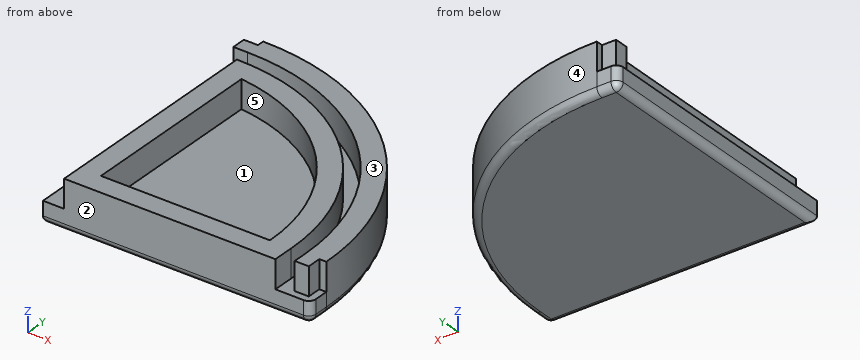
from build123d import *

# Parameters (mm, degrees)
BOSS_EXTRUDE1_DEPTH = 1.5
BOSS_EXTRUDE2_DEPTH = 2
FILETE1_R           = 0.5


with BuildPart() as part:
    # Sketch1 → Boss-Extrude1 (new body)
    with BuildSketch(Plane.XY):
        with BuildLine():
            Line((0, 0), (0, 19))
            Line((0, 19), (1.5, 19))
            ThreePointArc((1.5, 19), (13.874368671, 13.874368671), (19, 1.5))
            Line((19, 1.5), (19, 0))
            Line((19, 0), (0, 0))
        make_face()
    extrude(amount=BOSS_EXTRUDE1_DEPTH)

    # Sketch2 → Boss-Extrude2 (add)
    # profile 1 of 2: a face of its own
    with BuildSketch(Plane.XY.offset(1.5)):
        with BuildLine():
            Line((1.5, 19), (1.5, 18.5))
            Line((1.5, 18.5), (0.5, 18.5))
            Line((0.5, 18.5), (0.5, 17.5))
            Line((0.5, 17.5), (1.5, 17.5))
            ThreePointArc((1.5, 17.5), (12.813708499, 12.813708499), (17.5, 1.5))
            Line((17.5, 1.5), (17.5, 0.5))
            Line((17.5, 0.5), (18.5, 0.5))
            Line((18.5, 0.5), (18.5, 1.5))
            Line((18.5, 1.5), (19, 1.5))
            ThreePointArc((19, 1.5), (13.874368671, 13.874368671), (1.5, 19))
        make_face()
    # profile 2 of 2: a face of its own
    with BuildSketch(Plane.XY.offset(1.5)):
        with BuildLine():
            Line((1.5, 16.5), (1.5, 0))
            Line((1.5, 0), (16.5, 0))
            Line((16.5, 0), (16.5, 1.5))
            ThreePointArc((16.5, 1.5), (12.106601718, 12.106601718), (1.5, 16.5))
        make_face()
        with BuildLine():
            Line((3, 14.916407865), (3, 1.5))
            Line((3, 1.5), (15, 1.5))
            ThreePointArc((15, 1.5), (11.562305899, 10.5), (3, 14.916407865))
        make_face(mode=Mode.SUBTRACT)
    extrude(amount=BOSS_EXTRUDE2_DEPTH)

    # Filete1
    filete1_edges = [part.edges().sort_by_distance(p)[0] for p in [
        (0, 9.5, 0),
        (0.75, 19, 0),
        (13.874368671, 13.874368671, 0),
        (19, 0.75, 0),
        (9.5, 0, 0),
        (0, 19, 0.75),
        (19, 0, 0.75),
    ]]
    fillet(filete1_edges, radius=FILETE1_R)


solid = part.part
Design review of the part built by this model. Coordinates are the model's own, in mm. Face numbers are marked on the shaded views. A direction names the side the tool comes from. Round coordinates to 2 decimals unless told otherwise and drop trailing zeros. Write each loop counter-clockwise with the first axis right and the second up, starting at its lowest first coordinate (ties: lowest second). Pieces come first, ordered by that corner, then holes. Notation, with made-up numbers: (-9, -34.75) - (20, -34.75) arc R18 cw to (20, -18.75) - close; hole circle Ø10 at (-12, 27.5). An arc over 180 degrees is marked (long way). Return JSON: item names as keys, results as strings. Group by question number.
Item 1: Insertion check: P1, Ø0.6, axis at y = 7, z = 2.5, coming from the -X side; P2, Ø1.6, axis at y = 10, z = 2.5, coming from the +X side; P3, Ø1, axis at x = 8, z = 1.5, coming from the +Y side. Each pin has a flat end and moves straight along its axis. Give the tip position at first contact, or say it passes through.
Item 2: Machinability: for the marked faces 4 and 5, which of the approach directions +Z, -Z, +X, -X, +Y, -Y give a long, thin tool a straight path to every point of the face, cutting with its end or side? Answer none if there is none.
Item 3: The part is to be moulded in two halves that separate along Y. For the marked faces 1, 2 and 3, say which applies: pulls with the +Y half, pulls with the -Y half, needs draft (parallel to the pull), parting line crosses it, or undercut.
Item 4: We need section A-A on z = 1.75. Write out the cut boundary in (x, y).
Item 5: For probe 1 along Y at (x, z) = (13.5, 3); probe 2 along X at (y, z) = (6, 2.05); probe 3 along Y at (x, z) = (11.5, 2.2), list the stretches that pass through material, from the lowest coordinate up. Write a range as [from, to].
Model answer:
{
 "1": {"P1": "stops at x = 1.5", "P2": "stops at x = 17.21", "P3": "stops at y = 17.94"},
 "2": {"face 4": "+Z, -Z, +X, +Y", "face 5": "+Z"},
 "3": {"face 1": "undercut", "face 2": "pulls with the -Y half", "face 3": "needs draft"},
 "4": {"outline": "(0.5, 17.5) - (1.5, 17.5) arc R16 cw to (17.5, 1.5) - (17.5, 0.5) - (18.5, 0.5) - (18.5, 1.5) - (19, 1.5) arc R17.5 ccw to (1.5, 19) - (1.5, 18.5) - (0.5, 18.5) - close; (1.5, 0) - (16.5, 0) - (16.5, 1.5) arc R15 ccw to (1.5, 16.5) - close; hole (3, 1.5) - (15, 1.5) arc R13.5 ccw to (3, 14.92) - close"},
 "5": {"probe 1": "y = [0, 1.5], [7.68, 10.5], [12.08, 14.24]", "probe 2": "x = [1.5, 3], [14.23, 15.81], [16.85, 18.41]", "probe 3": "y = [0, 1.5], [10.57, 12.68], [13.99, 15.86]"}
}
